Geometry: final body of the model. Coordinates: model frame, mm. A direction names the side the tool comes from. Give positions to 0.01 mm unless a question says otherwise; leave off trailing zeros. Order: outer loops, then holes, each group sorted by start corner. A loop starts at its lowest first (then second) coordinate and runs counter-clockwise, first axis right, second up. Notation, with made-up numbers: (-19.5, 36.25) -> (4.5, 36.25) arc R19 cw to (4.5, 47.25) -> close; hole circle Ø8 at (74.25, -21). An arc over 180 degrees is marked (long way). Write item = value, one per line.
```python
from build123d import *

# Parameters (mm, degrees)
BOSS_EXTRUDE1_DEPTH = 12.7
SKETCH1_5_R         = 2.6035
BOSS_EXTRUDE2_DEPTH = 4.826
SKETCH2_R           = 3.81
CUT_EXTRUDE1_DEPTH  = 50.038


with BuildPart() as part:
    # Sketch1 → Boss-Extrude1 (new, symmetric)
    with BuildSketch(Plane(origin=(0, 0, 0), x_dir=(1, 0, 0), z_dir=(0, 1, 0))):
        with BuildLine():
            Line((-23.495, 17.749485254), (-23.495, -39.400514746))
            Line((-23.495, -39.400514746), (0, -39.400514746))
            Line((0, -39.400514746), (0, -33.050514746))
            ThreePointArc((0, -33.050514746), (-13.273575299, -2.418042558), (-3.175, 29.402625733))
            Line((-3.175, 29.402625733), (-3.175, 38.444242963))
            Line((-3.175, 38.444242963), (-8.255, 38.444242963))
            Line((-8.255, 38.444242963), (-23.495, 17.749485254))
        make_face()
    extrude(amount=BOSS_EXTRUDE1_DEPTH, both=True)

    # Sketch1<5> → Boss-Extrude2 (add, symmetric)
    with BuildSketch(Plane(origin=(0, 0, 0), x_dir=(1, 0, 0), z_dir=(0, 1, 0))):
        Polygon((0, -39.400514746), (-23.495, -39.400514746), (-35.052, -57.180514746), (-35.052, -77.500514746), (0, -77.500514746), align=None)
        with Locations(Location((-28.702, -64.800514746, 0), (0, 0, 270))):
            Circle(SKETCH1_5_R, mode=Mode.SUBTRACT)
        with Locations(Location((-8.382, -64.800514746, 0), (0, 0, 270))):
            Circle(SKETCH1_5_R, mode=Mode.SUBTRACT)
    extrude(amount=BOSS_EXTRUDE2_DEPTH, both=True)

    # Sketch2 → Cut-Extrude1 (cut)
    with BuildSketch(Plane.XY.offset(77.500514746)):
        Circle(SKETCH2_R)
    extrude(amount=-CUT_EXTRUDE1_DEPTH, mode=Mode.SUBTRACT)


solid = part.part
```
1) Line query: line 1 (Z direction, x = -9.5, y = 3.5); line 2 (Y direction, x = -24, z = 57.5); line 3 (Z direction, x = -28, y = -3). Output: solid intervals per line, ascending. Write a range as from..to.
Check sheet entries:
line_1 = -36.75..-18.72, 18.72..62.45, 67.15..77.5
line_2 = -4.83..4.83
line_3 = 46.33..62.29, 67.31..77.5
2) Section query C-C (y = 9.25). Output: boundary loops of the cut face in (x, z) (3 decimals).
Check sheet entries:
outline = (-23.495, -17.749) -> (-8.255, -38.444) -> (-3.175, -38.444) -> (-3.175, -29.403) arc R47.625 cw to (0, 33.051) -> (0, 39.401) -> (-23.495, 39.401) -> close
3) Mould query, pull axis X, two halves, no side actions, for faces 1 (the face through (-15.8, 0.2, -28.2)), 2 (the face through (0, -4.6, 45.5)), 3 (the face through (-31.012, -0.068, 66.002)), 4 (the face through (-15, -12.7, 9)). Classes: +X half, -X half, draft (parallel to the pull), parting line (faces both ways), or undercut.
Check sheet entries:
face_1 = -X half
face_2 = +X half
face_3 = undercut
face_4 = draft
4) Section query D-D (y = 0). Count the separate pieces of the cut face and the enclosed holes in it, plus the area to 3 significant figures.
Check sheet entries:
separate_pieces = 1
enclosed_holes = 2
area = 2,050 mm²
5) Reachability of faces 5 (the face through (-3.175, 0, -34)), 6 (the face through (-3.81, 0.08, 53.38)), 7 (the face through (-23.495, 0, 10)), 8 (the face through (-18, 4.826, 58)), 9 (the face through (-12, -9, 39.401)) from +Z, -Z, +X, -X, +Y, -Y: full face, straight path, thin tool, end or side. Return the list, or none.
Check sheet entries:
face_5 = -Z, +X, +Y, -Y
face_6 = +Z, +X
face_7 = -Z, -X, +Y, -Y
face_8 = +Z, +X, -X, +Y
face_9 = +Z, +X, -X, -Y
6) Section query A-A (z = 66). Output: boundary loops of the cut face in (x, y), plus the area to 3 significant figures.
Check sheet entries:
outline = (-35.05, -4.83) -> (-31.01, -4.83) -> (-31.01, 4.83) -> (-35.05, 4.83) -> close; (-26.39, -4.83) -> (-10.69, -4.83) -> (-10.69, 4.83) -> (-26.39, 4.83) -> close; (-6.07, -4.83) -> (0, -4.83) -> (0, -3.81) arc R3.81 cw to (0, 3.81) -> (0, 4.83) -> (-6.07, 4.83) -> close
area = 226 mm²
7) First-contact query: P1, Ø2.5, axis at y = -2.5, z = -35, coming from the +X side (3 decimals); P2, Ø8, axis at x = -18.5, y = -4, coming from the -Z side; P3, Ø4, axis at x = -10, y = 9.5, coming from the +Z side; P4, Ø3, axis at x = -8.38, z = 64.8, coming from the -Y side. Flat tips, straight axial feed; report the tip coordinate or a pass-through.
Check sheet entries:
P1 = -3.175
P2 = -29.96
P3 = 39.4
P4 = through
8) Section query B-B (x = -27.5). Output: boundary loops of the cut face in (y, z), plus the area to 3 significant figures.
Check sheet entries:
outline = (-4.83, 45.56) -> (4.83, 45.56) -> (4.83, 62.49) -> (-4.83, 62.49) -> close; (-4.83, 67.11) -> (4.83, 67.11) -> (4.83, 77.5) -> (-4.83, 77.5) -> close
area = 264 mm²
